Model file for the job. Use its own axes, mm. A direction names the side the tool comes from. Round coordinates to 2 decimals unless told otherwise and drop trailing zeros. Loops run counter-clockwise (first coordinate to the right, second up) from the corner with the lowest first, then second, coordinate; pieces in that order, holes last. Notation, with made-up numbers: M -0.75,61 L 35.25,61 A30 ccw 35.25,85 Z; hole C 38,-30 d2. An arc over 180 degrees is marked long. Answer in a Markdown table with one row per item.
from build123d import *

# Parameters (mm, degrees)
EXTRUDE_1_DEPTH = 12.5
SKETCH_3_R      = 8.7
EXTRUDE_2_DEPTH = 85
EXTRUDE_3_DEPTH = 9.5


with BuildPart() as part:
    # 草图1 → 旋转1 (revolve)
    with BuildSketch(Plane.XY, mode=Mode.PRIVATE) as revolve_1_sk:
        Polygon((-8, 0), (-8, 4.3865), (-7.3865, 5), (0, 5), (0, 0), align=None)
    revolve(revolve_1_sk.sketch.rotate(Axis((0, 0, 0), (-1, 0, 0)), 270), axis=Axis((0, 0, 0), (-1, 0, 0)))

    # 草图2 → 凸台-拉伸1 (add)
    with BuildSketch(Plane(origin=(0, 0, 0), x_dir=(0, 0, -1), z_dir=(1, 0, 0))):
        with BuildLine():
            Line((-4.034538387, -9.15), (4.034538387, -9.15))
            ThreePointArc((4.034538387, -9.15), (7.071067812, -7.071067812), (9.15, -4.034538387))
            Line((9.15, -4.034538387), (9.15, 4.034538387))
            ThreePointArc((9.15, 4.034538387), (7.071067812, 7.071067812), (4.034538387, 9.15))
            Line((4.034538387, 9.15), (-4.034538387, 9.15))
            ThreePointArc((-4.034538387, 9.15), (-7.071067812, 7.071067812), (-9.15, 4.034538387))
            Line((-9.15, 4.034538387), (-9.15, -4.034538387))
            ThreePointArc((-9.15, -4.034538387), (-7.071067812, -7.071067812), (-4.034538387, -9.15))
        make_face()
    extrude(amount=EXTRUDE_1_DEPTH)

    # 草图3 → 凸台-拉伸2 (add)
    with BuildSketch(Plane(origin=(12.5, 0, 0), x_dir=(0, 0, -1), z_dir=(1, 0, 0))):
        Circle(SKETCH_3_R)
    extrude(amount=EXTRUDE_2_DEPTH)

    # 草图4 → 凸台-拉伸3 (add)
    with BuildSketch(Plane(origin=(97.5, 0, 0), x_dir=(0, 0, -1), z_dir=(1, 0, 0))):
        with BuildLine():
            Line((-4.034538387, -9.15), (4.034538387, -9.15))
            ThreePointArc((4.034538387, -9.15), (7.071067812, -7.071067812), (9.15, -4.034538387))
            Line((9.15, -4.034538387), (9.15, 4.034538387))
            ThreePointArc((9.15, 4.034538387), (7.071067812, 7.071067812), (4.034538387, 9.15))
            Line((4.034538387, 9.15), (-4.034538387, 9.15))
            ThreePointArc((-4.034538387, 9.15), (-7.071067812, 7.071067812), (-9.15, 4.034538387))
            Line((-9.15, 4.034538387), (-9.15, -4.034538387))
            ThreePointArc((-9.15, -4.034538387), (-7.071067812, -7.071067812), (-4.034538387, -9.15))
        make_face()
    extrude(amount=EXTRUDE_3_DEPTH)

    # 草图5 → 切除-旋转1 (revolve, cut)
    with BuildSketch(Plane.XY, mode=Mode.PRIVATE) as cut_revolve_1_sk:
        Polygon((8, 2.456616994), (5.933, 3.65), (5.933, 8.717), (5.5, 9.15), (8, 9.15), align=None)
    revolve(cut_revolve_1_sk.sketch.rotate(Axis((8, 9.15, 0), (0, -1, 0)), 90), axis=Axis((8, 9.15, 0), (0, -1, 0)), mode=Mode.SUBTRACT)

    # 草图6 → 切除-旋转2 (revolve, cut)
    with BuildSketch(Plane.XY, mode=Mode.PRIVATE) as cut_revolve_2_sk:
        Polygon((102, 2.456616994), (99.933, 3.65), (99.933, 8.717), (99.5, 9.15), (102, 9.15), align=None)
    revolve(cut_revolve_2_sk.sketch.rotate(Axis((102, 9.15, 0), (0, -1, 0)), 90), axis=Axis((102, 9.15, 0), (0, -1, 0)), mode=Mode.SUBTRACT)

    # 草图7 → 切除-旋转3 (revolve, cut)
    with BuildSketch(Plane.XY, mode=Mode.PRIVATE) as cut_revolve_3_sk:
        Polygon((-8, 0), (-8, 2.5), (12.5, 2.5), (12.5, 8), (77.5, 8), (77.5, 0), align=None)
    revolve(cut_revolve_3_sk.sketch.rotate(Axis((50, 0, 0), (-1, 0, 0)), 270), axis=Axis((50, 0, 0), (-1, 0, 0)), mode=Mode.SUBTRACT)


solid = part.part
1. Saw through at A-A (y = 0). Write the cut outline in (x, z).
Verdict:
| item | result |
|---|---|
| outline | M -8,-4.39 L -7.39,-5 L 0,-5 L 0,-9.15 L 12.5,-9.15 L 12.5,-8.7 L 97.5,-8.7 L 97.5,-9.15 L 107,-9.15 L 107,9.15 L 97.5,9.15 L 97.5,8.7 L 12.5,8.7 L 12.5,9.15 L 0,9.15 L 0,5 L -7.39,5 L -8,4.39 L -8,2.5 L 12.5,2.5 L 12.5,8 L 77.5,8 L 77.5,-8 L 12.5,-8 L 12.5,-2.5 L -8,-2.5 Z |
2. Wall check: probe 1 along X at (y, z) = (6, 0); probe 2 along X at (y, z) = (-5.5, -4.25); probe 3 along X at (y, z) = (4.8, 0). Give the ranges that are in metal, low to high.
Verdict:
| item | result |
|---|---|
| probe 1 | x = 0 to 5.93, 10.07 to 12.5, 77.5 to 99.93, 104.07 to 107 |
| probe 2 | x = 0 to 12.5, 77.5 to 107 |
| probe 3 | x = -7.59 to 5.93, 10.07 to 12.5, 77.5 to 99.93, 104.07 to 107 |
3. Saw through at D-D (x = 89). Write the cut outline in (y, z), and give its area (3 significant figures).
Verdict:
| item | result |
|---|---|
| outline | C 0,0 d17.4 |
| area | 238 mm² |
4. Tool access for faces 1 (the cylindrical face through (6.16, 7.11, 7.03)), 2 (the cylindrical face through (103.743, 6.219, -1.111)), 3 (the cylindrical face through (-3.64, -4.88, -1.08)), 4 (the flat face through (102, 0, 9.15)), 5 (the cylindrical face through (54.405, -8.493, 1.886)): list every direction of +Z, -Z, +X, -X, +Y, -Y with a clear straight run to the whole face (end or side of a thin tool).
Verdict:
| item | result |
|---|---|
| face 1 | +Z, +X, -X, +Y |
| face 2 | +Y |
| face 3 | -X |
| face 4 | +Z, +X, -X, +Y, -Y |
| face 5 | none |
5. Pin check, flat tips, straight feed: pin 1 (10 mm diameter, centred on x = 91.5, y = -2.5, fed in from +Z); pin 2 (2 mm diameter, centred on y = -5.5, z = 3.5, fed in from -X); pin 3 (3 mm diameter, centred on y = 0, z = 0, fed in from -X). Stop position of each tip, or through.
Verdict:
| item | result |
|---|---|
| pin 1 | stops at z = 8.7 |
| pin 2 | stops at x = 0 |
| pin 3 | stops at x = 77.5 |
6. Saw through at C-C (x = 17). Write the cut outline in (y, z).
Verdict:
| item | result |
|---|---|
| outline | C 0,0 d17.4; hole C 0,0 d16 |
7. Mould opens along X. For faces 6 (the flat face through (0, -4, -4)), 7 (the conical face through (101.65, 2.664, 0.078)), 8 (the cylindrical face through (5.982, 6.219, 0.448)), 9 (the cylindrical face through (2.39, -2.44, -0.54)) say: +X half, -X half, draft (parallel to the pull), parting line (faces both ways), or undercut.
Verdict:
| item | result |
|---|---|
| face 6 | -X half |
| face 7 | undercut |
| face 8 | undercut |
| face 9 | draft |
8. Saw through at B-B (z = -6.75). Write the cut outline in (x, y), and give its area (3 significant figures).
Verdict:
| item | result |
|---|---|
| outline | M 0,-7.38 L 12.5,-7.38 L 12.5,-5.49 L 97.5,-5.49 L 97.5,-7.38 L 107,-7.38 L 107,7.38 L 97.5,7.38 L 97.5,5.49 L 12.5,5.49 L 12.5,7.38 L 0,7.38 Z; hole M 12.5,-4.29 L 77.5,-4.29 L 77.5,4.29 L 12.5,4.29 Z |
| area | 700 mm² |
